Check sheet for the drawn part. Datum: minimum x, y, z corner. Units: mm. A direction names the side the tool comes from. Give positions to 0.01 mm unless a question says otherwise; leave off trailing zeros. Write each loop counter-clockwise with the first axis right and the second up, starting at its lowest first coordinate (ties: lowest second). Pieces come first, ordered by that corner, then holes.
(1) Cross-section at D-D (x = 82). Record the boundary of the cut face in (y, z) (1 decimal).
(2) Cross-section at B-B (y = 225.5). Record the boundary of the cut face in (x, z), and give its area (3 significant figures).
(3) Thickness scan on line 1 along Y through (x, z) = (7, 29.5); line 2 along Y through (x, z) = (23.5, 23.5); line 3 along Y through (x, z) = (86, 40.5). Record the ranges inside material, lowest first.
(4) Cross-section at C-C (z = 65). Record the boundary of the cut face in (x, y).
(5) Depth check by flat-ended pin: P1, Ø24, axis at x = 53.13, y = 90.6, coming from the +Z side; P2, Ø6, axis at x = 77.5, y = 74.5, coming from the -Z side. Enter the tip coordinate at first touch or a pass-through.
(6) Cross-section at A-A (x = 11). Record the boundary of the cut face in (y, z) (1 decimal), and give its area (3 significant figures).
(7) Mould release check, pull along Y, two halves, no side actions. Record for the marked faces 6, 7 and 8: +Y half, -Y half, draft (parallel to the pull), parting line (faces both ways), or undercut.
(8) Tool access check on the marked faces 1, 2, 3, 4 and 5. Record the directions out of +Z, -Z, +X, -X, +Y, -Y that give a thin tool (end or side, any length) a straight path to the whole face; none if there is none.
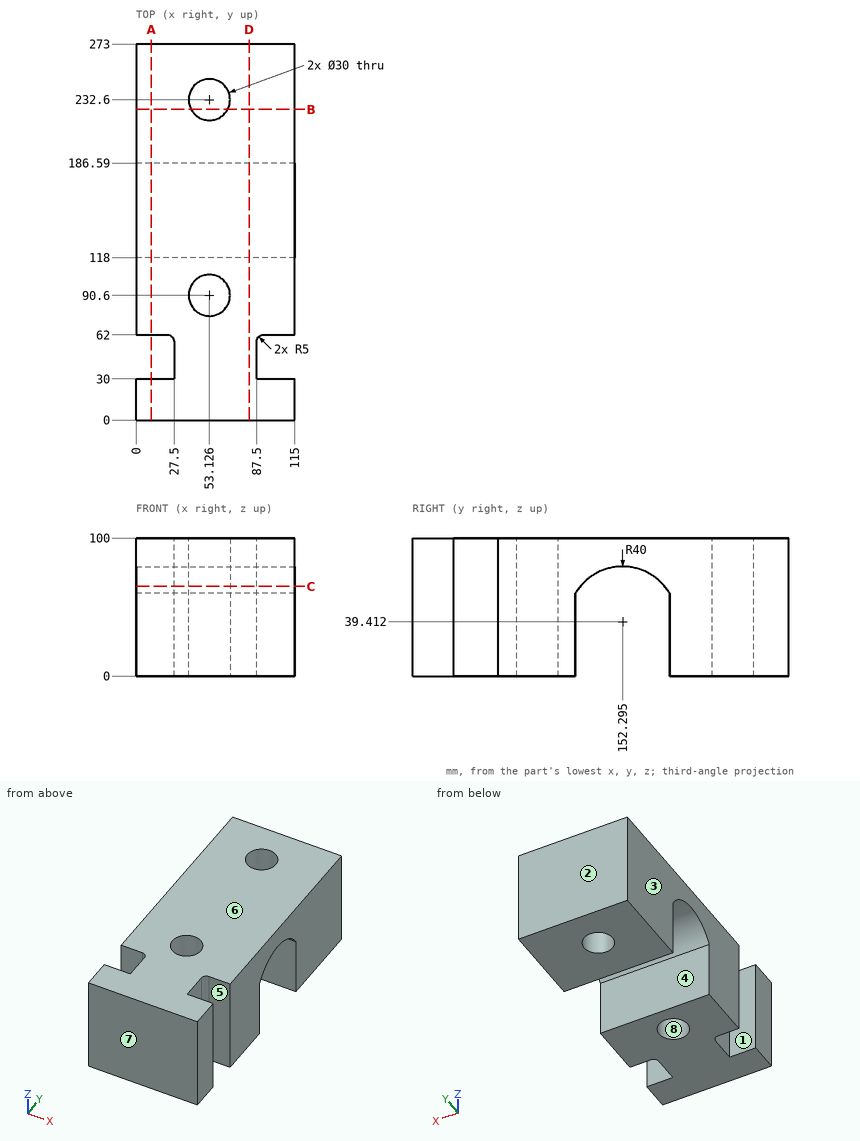
Reply:
1. outline: (0, 0) - (118, 0) - (118, 60) arc R40 cw to (186.6, 60) - (186.6, 0) - (273, 0) - (273, 100) - (0, 100) - close
2. outline: (0, 0) - (39.91, 0) - (39.91, 100) - (0, 100) - close; (66.34, 0) - (115, 0) - (115, 100) - (66.34, 100) - close
2. area: 8,860 mm2
3. line 1: y = 0 to 30, 62 to 118, 186.59 to 273
3. line 2: y = 0 to 30, 61.9 to 118, 186.59 to 273
3. line 3: y = 0 to 118, 186.59 to 273
4. outline: (0, 0) - (115, 0) - (115, 30) - (87.5, 30) - (87.5, 57) arc R5 cw to (92.5, 62) - (115, 62) - (115, 121.55) - (0, 121.55) - (0, 62) - (22.5, 62) arc R5 cw to (27.5, 57) - (27.5, 30) - (0, 30) - close; (0, 183.04) - (115, 183.04) - (115, 273) - (0, 273) - close; hole circle Ø30 at (53.13, 90.6); hole circle Ø30 at (53.13, 232.6)
5. P1: passes through
5. P2: stops at z = 0
6. outline: (0, 0) - (30, 0) - (30, 100) - (0, 100) - close; (62, 0) - (118, 0) - (118, 60) arc R40 cw to (186.6, 60) - (186.6, 0) - (273, 0) - (273, 100) - (62, 100) - close
6. area: 19,000 mm2
7. face 6: draft
7. face 7: -Y half
7. face 8: undercut
8. face 1: +Z, -Z, -X
8. face 2: +Z, -Z, +X, -X, +Y
8. face 3: +Z, -Z, -X, +Y, -Y
8. face 4: -Z, +X, -X
8. face 5: +Z, -Z, +X
